Geometry check sheet. Reference: the model listing, model coordinates, mm. A direction names the side the tool comes from. Give positions to 0.01 mm unless a question says otherwise; leave off trailing zeros. Order: outer loops, then holes, each group sorted by start corner. A loop starts at its lowest first (then second) coordinate and runs counter-clockwise, first axis right, second up.
from build123d import *

# Parameters (mm, degrees)
SKETCH_1_R          = 70
SKETCH_1_R_2        = 37.5
EXTRUDE_1_DEPTH     = 30
SKETCH_2_R          = 45
CUT_EXTRUDE_1_DEPTH = 1
CHAMFER_1_SIZE      = 1


with BuildPart() as part:
    # 草图1 → 凸台-拉伸1 (new body)
    with BuildSketch(Plane.XY):
        Circle(SKETCH_1_R)
        Circle(SKETCH_1_R_2, mode=Mode.SUBTRACT)
    extrude(amount=EXTRUDE_1_DEPTH)

    # 草图2 → 切除-拉伸1 (cut)
    with BuildSketch(Plane.XY.offset(30)):
        Circle(SKETCH_2_R)
    extrude(amount=-CUT_EXTRUDE_1_DEPTH, mode=Mode.SUBTRACT)

    # 倒角1
    chamfer_1_edges = [part.edges().sort_by_distance(p)[0] for p in [
        (-37.5, 0, 29),
    ]]
    chamfer(chamfer_1_edges, length=CHAMFER_1_SIZE)


solid = part.part
Item 1: Scan lines: L1, parallel to Y at x = 0, z = 8.75; L2, parallel to Y at x = 0, z = 29.6; L3, parallel to X at y = 30, z = 20. Record each from-to range of solid material in increasing order.
Reported:
L1: y = -70 to -37.5, 37.5 to 70
L2: y = -70 to -45, 45 to 70
L3: x = -63.25 to -22.5, 22.5 to 63.25
Item 2: Gauge pin test, flat ends, axial feed: pin 1 (1.5 mm diameter, centred on y = 51, z = 25.5, fed in from +X); pin 2 (4 mm diameter, centred on y = 4, z = 24.5, fed in from +X); pin 3 (1 mm diameter, centred on x = 4.5, y = -37.5, fed in from +Z); pin 4 (5 mm diameter, centred on x = -32.5, y = 5.5, fed in from -Z). Record the tip position at first contact, or that the pin passes through.
Reported:
pin 1: stops at x = 48.73
pin 2: stops at x = 69.97
pin 3: stops at z = 28.77
pin 4: passes through
Item 3: Sectioned sample at D-D (x = 58). Enter the section's corners in (y, z), and give its area (3 significant figures).
Reported:
outline: (-39.19, 0) - (39.19, 0) - (39.19, 30) - (-39.19, 30) - close
area: 2,350 mm2
Item 4: Sectioned sample at C-C (z = 13.75). Enter the section's corners in (x, y), and give its area (3 significant figures).
Reported:
outline: circle Ø140 at (0, 0); hole circle Ø75 at (0, 0)
area: 11,000 mm2
Item 5: Draft check along X on faces 1 (the flat face through (33.1, 20.2, 29)), 2 (the cylindrical face through (-55.55, -42.594, 14.79)), 3 (the flat face through (-1, -46, 30)). Enter one of: released by +X, released by -X, zero draft, split by the parting line, or undercut.
Reported:
face 1: undercut
face 2: split by the parting line
face 3: zero draft
Item 6: Set-up check for faces 4 (the cylindrical face through (20.765, -39.923, 29.507)), 5 (the cylindrical face through (-4.88, 37.18, 13.8)): record each of +Z, -Z, +X, -X, +Y, -Y from which the full face is reachable in a straight line by a thin tool's end or side.
Reported:
face 4: +Z
face 5: +Z, -Z
Item 7: Sectioned sample at A-A (y = 0). Enter the section's corners in (x, z), and give its area (3 significant figures).
Reported:
outline: (-70, 0) - (-37.5, 0) - (-37.5, 28) - (-38.5, 29) - (-45, 29) - (-45, 30) - (-70, 30) - close; (37.5, 0) - (70, 0) - (70, 30) - (45, 30) - (45, 29) - (38.5, 29) - (37.5, 28) - close
area: 1,930 mm2
